```python
from build123d import *

# Parameters (mm, degrees)
SKETCH1_W           = 110
SKETCH1_H           = 40
SKETCH1_R           = 3.5
BOSS_EXTRUDE1_DEPTH = 5
CHAMFER1_SIZE       = 3


with BuildPart() as part:
    # Sketch1 → Boss-Extrude1 (new body)
    with BuildSketch(Plane.XY):
        Rectangle(SKETCH1_W, SKETCH1_H)
        with Locations((-35, 0)):
            Circle(SKETCH1_R, mode=Mode.SUBTRACT)
        with Locations((35, 0)):
            Circle(SKETCH1_R, mode=Mode.SUBTRACT)
    extrude(amount=BOSS_EXTRUDE1_DEPTH)

    # Chamfer1
    chamfer1_edges = [part.edges().sort_by_distance(p)[0] for p in [
        (55, -20, 2.5),
        (55, 20, 2.5),
        (-55, 20, 2.5),
        (-55, -20, 2.5),
    ]]
    chamfer(chamfer1_edges, length=CHAMFER1_SIZE)


solid = part.part
```
Here's how the part is built. I have some questions about the finished solid (model axes, mm). Coordinates: 2 decimals unless noted, no trailing zeros. Write each loop counter-clockwise with the first axis right and the second up, starting at its lowest first coordinate (ties: lowest second). Pieces come first, ordered by that corner, then holes. Notation, with made-up numbers: (-11, 78) - (44, 78) arc R25 cw to (44, 107) - close; hole circle Ø11 at (-31, 86). An arc over 180 degrees is marked (long way). One line per item, written item: value.
1) Suppose I cut it at A-A on z = 2.2. Write out the boundary of the cut face in (x, y), and give its area (3 significant figures).
Model answer:
outline: (-55, -17) - (-52, -20) - (52, -20) - (55, -17) - (55, 17) - (52, 20) - (-52, 20) - (-55, 17) - close; hole circle Ø7 at (-35, 0); hole circle Ø7 at (35, 0)
area: 4,310 mm²
2) I'm going to push a flat-ended pin straight in: P1, Ø5.5, axis at x = 35, y = 0, coming from the +Z side. Where does the tip first touch, or does it pass through?
Model answer:
P1: passes through
3) I need wall thicknesses on line 1 along Y through (x, z) = (35, 3.9); line 2 along X through (y, z) = (-0.5, 3.4); line 3 along Y through (x, z) = (-33.5, 1.15). Which ranges of each line are inside material? Lowest first, please.
Model answer:
line 1: y = -20 to -3.5, 3.5 to 20
line 2: x = -55 to -38.46, -31.54 to 31.54, 38.46 to 55
line 3: y = -20 to -3.16, 3.16 to 20
4) We'd pull the mould along X, two halves only. Please class faces 1 (the flat face through (-1, 20, 2)), 2 (the flat face through (-53, 19, 2)), 3 (the cylindrical face through (-38.497, 0.154, 2.465)): pulls with the +X half, pulls with the -X half, needs draft (parallel to the pull), parting line crosses it, or undercut.
Model answer:
face 1: needs draft
face 2: pulls with the -X half
face 3: undercut
5) Suppose I cut it at B-B on y = 0. Write out the boundary of the cut face in (x, z).
Model answer:
outline: (-55, 0) - (-38.5, 0) - (-38.5, 5) - (-55, 5) - close; (-31.5, 0) - (31.5, 0) - (31.5, 5) - (-31.5, 5) - close; (38.5, 0) - (55, 0) - (55, 5) - (38.5, 5) - close
6) Suppose I cut it at C-C on x = -35. Write out the boundary of the cut face in (y, z), and give its area (3 significant figures).
Model answer:
outline: (-20, 0) - (-3.5, 0) - (-3.5, 5) - (-20, 5) - close; (3.5, 0) - (20, 0) - (20, 5) - (3.5, 5) - close
area: 165 mm²
